Could you check a few things on this model? Use its own coordinates, in mm. Face numbers are marked on the shaded views. A direction names the side the tool comes from. Coordinates: 2 decimals unless noted, no trailing zeros. Order: outer loops, then holes, each group sorted by start corner. A loop starts at its lowest first (then second) coordinate and runs counter-clockwise, first axis right, second up. Notation, with made-up numbers: (62.5, 64.5) -> (121.5, 64.5) arc R31 cw to (121.5, 96.5) -> close; hole circle Ø3 at (-24, 75). An arc over 180 degrees is marked (long way). Put each result on its own line as item: value. Start each with the question number.
Q1. If we section it at C-C (x = 0.75): Please give me the cut outline in (y, z).
Q2. If we section it at D-D (y = -2.25): Please give me the cut outline in (x, z).
Q3. If we section it at A-A (x = -11): Please give me the cut outline in (y, z).
Q4. Please list where these lines run through material, in increasing order: line 1 along Z through (x, y) = (-11, -2.1); line 2 along X through (y, z) = (0.05, 9.5); line 3 along Z through (x, y) = (-2.25, -0.85).
Q5. For the marked faces 3 and 4, which set-ups out of +Z, -Z, +X, -X, +Y, -Y let a thin tool reach every point of the face, with its end or its side?
Q6. If we section it at B-B (y = 0): Please give me the cut outline in (x, z), and give its area (3 significant figures).
Q7. We'd pull the mould along X, two halves only. Please class the marked faces 1 and 2: +X half, -X half, draft (parallel to the pull), parting line (faces both ways), or undercut.
Q8. Will these pins go through, and if not, where does the flat tip stop? pin 1 (2 mm diameter, centred on x = -13.5, z = -5.5, fed in from +Y); pin 2 (1.2 mm diameter, centred on y = -2, z = 3, fed in from +X); pin 3 (2 mm diameter, centred on x = -2, y = 2.5, fed in from -Z); pin 4 (1.8 mm diameter, centred on x = 0, y = 0, fed in from +Z).
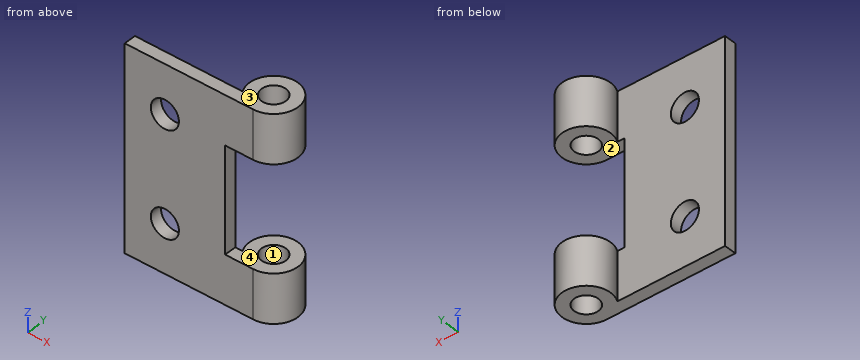
from build123d import *

# Parameters (mm, degrees)
SKETCH_1_R          = 1.5
EXTRUDE_1_DEPTH     = 12.5
CUT_EXTRUDE_1_DEPTH = 6.5
SKETCH_3_R          = 1.75
CUT_EXTRUDE_2_DEPTH = 21.796634343


with BuildPart() as part:
    # 草图1 → 凸台-拉伸1 (new, symmetric)
    with BuildSketch(Plane.XY):
        with BuildLine():
            Line((-2.598076211, -1.5), (-16, -1.5))
            Line((-16, -1.5), (-16, -3))
            Line((-16, -3), (0, -3))
            ThreePointArc((0, -3), (1.5, 2.598076211), (-2.598076211, -1.5))
        make_face()
        Circle(SKETCH_1_R, mode=Mode.SUBTRACT)
    extrude(amount=EXTRUDE_1_DEPTH, both=True)

    # 草图2 → 切除-拉伸1 (cut, symmetric)
    with BuildSketch(Plane.XY):
        with BuildLine():
            Line((-3.5, 0), (-3.5, -3))
            Line((-3.5, -3), (-1.802775638, -3))
            ThreePointArc((-1.802775638, -3), (3.046285831, 1.723410176), (-3.5, 0))
        make_face()
    extrude(amount=CUT_EXTRUDE_1_DEPTH, both=True, mode=Mode.SUBTRACT)

    # 草图3 → 切除-拉伸2 (cut, through all)
    with BuildSketch(Plane(origin=(0, -1.5, 0), x_dir=(1, 0, 0), z_dir=(0, 1, 0))):
        with Locations(Location((-11, 6.5, 0), (0, 0, 180))):
            Circle(SKETCH_3_R)
        with Locations((-11, -6.5)):
            Circle(SKETCH_3_R)
    extrude(amount=-CUT_EXTRUDE_2_DEPTH, mode=Mode.SUBTRACT)


solid = part.part
The answers:
1. outline: (-2.9, -12.5) -> (-1.3, -12.5) -> (-1.3, -6.5) -> (-2.9, -6.5) -> close; (-2.9, 6.5) -> (-1.3, 6.5) -> (-1.3, 12.5) -> (-2.9, 12.5) -> close; (1.3, -12.5) -> (2.9, -12.5) -> (2.9, -6.5) -> (1.3, -6.5) -> close; (1.3, 6.5) -> (2.9, 6.5) -> (2.9, 12.5) -> (1.3, 12.5) -> close
2. outline: (-16, -12.5) -> (1.98, -12.5) -> (1.98, -6.5) -> (-3.5, -6.5) -> (-3.5, 6.5) -> (1.98, 6.5) -> (1.98, 12.5) -> (-16, 12.5) -> close; hole circle Ø3.5 at (-11, -6.5); hole circle Ø3.5 at (-11, 6.5)
3. outline: (-3, -12.5) -> (-1.5, -12.5) -> (-1.5, -8.25) -> (-3, -8.25) -> close; (-3, -4.75) -> (-1.5, -4.75) -> (-1.5, 4.75) -> (-3, 4.75) -> close; (-3, 8.25) -> (-1.5, 8.25) -> (-1.5, 12.5) -> (-3, 12.5) -> close
4. line 1: -12.5 to -8.25, -4.75 to 4.75, 8.25 to 12.5
4. line 2: -3 to -1.5, 1.5 to 3
4. line 3: -12.5 to -6.5, 6.5 to 12.5
5. face 3: +Z, +X, -X, +Y, -Y
5. face 4: +X, +Y, -Y
6. outline: (-3, -12.5) -> (-1.5, -12.5) -> (-1.5, -6.5) -> (-3, -6.5) -> close; (-3, 6.5) -> (-1.5, 6.5) -> (-1.5, 12.5) -> (-3, 12.5) -> close; (1.5, -12.5) -> (3, -12.5) -> (3, -6.5) -> (1.5, -6.5) -> close; (1.5, 6.5) -> (3, 6.5) -> (3, 12.5) -> (1.5, 12.5) -> close
6. area: 36.0 mm^2
7. face 1: undercut
7. face 2: draft
8. pin 1: y = -1.5
8. pin 2: x = -3.5
8. pin 3: z = -12.5
8. pin 4: through
